Design review of the part built by this model. Coordinates are the model's own, in mm. Face numbers are marked on the shaded views. A direction names the side the tool comes from. Give positions to 0.01 mm unless a question says otherwise; leave off trailing zeros. Order: outer loops, then holes, each group sorted by start corner. A loop starts at its lowest first (then second) coordinate and runs counter-clockwise, first axis right, second up.
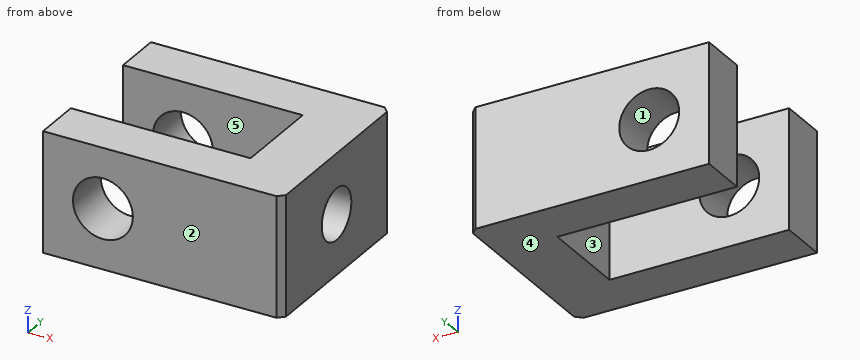
```python
from build123d import *

# Parameters (mm, degrees)
SKETCH_1_W                  = 40
SKETCH_1_H                  = 31
EXTRUDE_1_DEPTH             = 20
SKETCH_2_W                  = 30
SKETCH_2_H                  = 15
CUT_EXTRUDE_1_DEPTH         = 35.220141674
HOLE_WIZARD_10_0_10_1_D     = 10
HOLE_WIZARD_10_0_10_1_DEPTH = 8
HOLE_WIZARD_8_5_8_5_1_D     = 8.5
HOLE_WIZARD_8_5_8_5_1_DEPTH = 40
HOLE_WIZARD_10_0_10_2_D     = 10
CHAMFER_1_SIZE              = 1


with BuildPart() as part:
    # 草图1 → 凸台-拉伸1 (new body)
    with BuildSketch(Plane(origin=(0, 0, -10), x_dir=(-1, 0, 0), z_dir=(0, 0, -1))):
        with Locations((-3.03840481, 0)):
            Rectangle(SKETCH_1_W, SKETCH_1_H)
    extrude(amount=-EXTRUDE_1_DEPTH)

    # 草图2 → 切除-拉伸1 (cut, through all)
    with BuildSketch(Plane.XY.offset(10)):
        with Locations((-1.96159519, 0)):
            Rectangle(SKETCH_2_W, SKETCH_2_H)
    extrude(amount=-CUT_EXTRUDE_1_DEPTH, mode=Mode.SUBTRACT)

    # Ø10.0 (10) 直径孔1
    with Locations(Plane(origin=(0, -15.5, 0), x_dir=(-1, 0, 0), z_dir=(0, -1, 0))):
        with Locations((6.96159519, 0)):
            Hole(HOLE_WIZARD_10_0_10_1_D / 2, depth=HOLE_WIZARD_10_0_10_1_DEPTH)

    # Ø8.5 (8.5) 直径孔1
    with Locations(Plane(origin=(23.03840481, 0, 0), x_dir=(0, 0, -1), z_dir=(1, 0, 0))):
        with Locations((0, 0)):
            Hole(HOLE_WIZARD_8_5_8_5_1_D / 2, depth=HOLE_WIZARD_8_5_8_5_1_DEPTH)

    # Ø10.0 (10) 直径孔2 (through all)
    with Locations(Plane(origin=(0, 7.5, 0), x_dir=(-1, 0, 0), z_dir=(0, -1, 0))):
        with Locations((6.96159519, 0)):
            Hole(HOLE_WIZARD_10_0_10_2_D / 2)

    # 倒角1
    chamfer_1_edges = [part.edges().sort_by_distance(p)[0] for p in [
        (23.03840481, -15.5, 0),
        (23.03840481, 15.5, 0),
    ]]
    chamfer(chamfer_1_edges, length=CHAMFER_1_SIZE)


solid = part.part
```
1. Take a section at D-D (z = 8). State the section outline as (x, y) points, then the cut area to 3 significant figures.
Recorded:
outline: (-16.96, -15.5) - (22.04, -15.5) - (23.04, -14.5) - (23.04, 14.5) - (22.04, 15.5) - (-16.96, 15.5) - (-16.96, 7.5) - (13.04, 7.5) - (13.04, -7.5) - (-16.96, -7.5) - close
area: 789 mm2
2. Machinability: for the marked faces 4 and 5, which of the approach directions +Z, -Z, +X, -X, +Y, -Y give a long, thin tool a straight path to every point of the face, cutting with its end or side? Answer none if there is none.
Recorded:
face 4: -Z, +X, -X, +Y, -Y
face 5: +Z, -Z, -X
3. Take a section at C-C (z = 0). State the section outline as (x, y) points, then the cut area to 3 significant figures.
Recorded:
outline: (-16.96, -15.5) - (-11.96, -15.5) - (-11.96, -7.5) - (-16.96, -7.5) - close; (-16.96, 7.5) - (-11.96, 7.5) - (-11.96, 15.5) - (-16.96, 15.5) - close; (-1.96, -15.5) - (22.04, -15.5) - (23.04, -14.5) - (23.04, -4.25) - (13.04, -4.25) - (13.04, -7.5) - (-1.96, -7.5) - close; (-1.96, 7.5) - (13.04, 7.5) - (13.04, 4.25) - (23.04, 4.25) - (23.04, 14.5) - (22.04, 15.5) - (-1.96, 15.5) - close
area: 544 mm2
4. For line 1 along Y through (x, z) = (4.5, 2.5); line 2 along X through (y, z) = (2.5, -4); line 3 along Y through (x, z) = (16, 0), list the stretches that pass through material, from the lowest coordinate up.
Recorded:
line 1: y = -15.5 to -7.5, 7.5 to 15.5
line 2: x = 13.04 to 23.04
line 3: y = -15.5 to -4.25, 4.25 to 15.5
5. Take a section at A-A (y = 0). State the section outline as (x, z) points.
Recorded:
outline: (13.04, -10) - (23.04, -10) - (23.04, -4.25) - (13.04, -4.25) - close; (13.04, 4.25) - (23.04, 4.25) - (23.04, 10) - (13.04, 10) - close
6. For pin 1 (4.5 mm diameter, centred on y = 0, z = 2.5, fed in from -X); pin 2 (3 mm diameter, centred on x = -1, y = 4.5, fed in from -Z), all flat-tipped, find the tip position at first contact; note any pin that passes through.
Recorded:
pin 1: stops at x = 13.04
pin 2: passes through
7. Take a section at B-B (x = 1.5). State the section outline as (y, z) points.
Recorded:
outline: (-15.5, -10) - (-7.5, -10) - (-7.5, 10) - (-15.5, 10) - close; (7.5, -10) - (15.5, -10) - (15.5, 10) - (7.5, 10) - close
8. Draft analysis for pull direction X (two halves, no side actions). For the marked faces 1, 2 and 3, state which applies: pulls with the +X half, pulls with the -X half, needs draft (parallel to the pull), parting line crosses it, or undercut.
Recorded:
face 1: undercut
face 2: needs draft
face 3: pulls with the -X half
